The listing builds one solid part. Answer for the finished solid, in the listing's coordinates (mm). A direction names the side the tool comes from. Give positions to 0.01 mm unless a question says otherwise; leave off trailing zeros. Order: outer loops, then holes, each group sorted by start corner. A loop starts at its lowest first (then second) coordinate and runs counter-clockwise, first axis right, second up. Notation, with made-up numbers: (41, 6) - (92, 6) arc R22 cw to (92, 42) - close; hole circle Ø7 at (23, 59.25). An arc over 180 degrees is marked (long way). Write each question's results on one line, items separated by ' | '. Start each with the question number.
1. Which of the six approach directions +Z, -Z, +X, -X, +Y, -Y give full straight-line access (tool end or side, diameter ignored) to faces 5 (the face through (-6, -16.5, 0)), 6 (the face through (-6, 16.5, 0)), 7 (the face through (-430, 0.1, 16.4)), 8 (the face through (-6, 0, -16)), 9 (the face through (-440, 17.5, 0))?
2. Determine the mould class of faces 1 (the face through (440, 0, -17)), 2 (the face through (-6, 0, 16)), 3 (the face through (430, 0.1, 16.4)), 4 (the face through (-450, 0, 0)) for opening direction X: released by +X, released by -X, zero draft, split by the parting line, or undercut.
3. Find the intervals of material crossed by L1, parallel to Z at x = 400, y = 12.75; L2, parallel to Z at x = -311, y = -13; L3, parallel to Y at x = 29, z = -11, in increasing order.
4. Flat-ended cylindrical pins translate along their axes: pin 1 (6 mm diameter, centred on x = -67.5, z = 0.5, fed in from -Y); pin 2 (8 mm diameter, centred on x = 24.5, y = 10.5, fed in from -Z); pin 3 (1.5 mm diameter, centred on x = 83.5, y = 2, fed in from +Z). Find the tip coordinate at first contact, or state that the pin passes through.
5. Section A-A (z = -10) is taken. Give the vertices of the cut face in (x, y), and give its area (3 significant figures).
6. Section B-B (x = -164) is taken. Give the vertices of the cut face in (y, z), and give its area (3 significant figures).
from build123d import *

# Parameters (mm, degrees)
SKETCH_1_W                  = 900
SKETCH_1_H                  = 33
EXTRUDE_1_DEPTH             = 16
SKETCH_2_W                  = 34
SKETCH_2_H                  = 35
EXTRUDE_2_DEPTH             = 20
HOLE_WIZARD_4_5_4_5_1_D     = 4.5
HOLE_WIZARD_4_5_4_5_1_DEPTH = 10
HOLE_WIZARD_4_5_4_5_1_TIP   = 1.351936393


with BuildPart() as part:
    # 草图1 → 凸台-拉伸1 (new, symmetric)
    with BuildSketch(Plane.XY):
        Rectangle(SKETCH_1_W, SKETCH_1_H)
    extrude(amount=EXTRUDE_1_DEPTH, both=True)

    # 草图2 → 凸台-拉伸2 (add)
    with BuildSketch(Plane(origin=(450, 0, 0), x_dir=(0, 0, -1), z_dir=(1, 0, 0))):
        Rectangle(SKETCH_2_W, SKETCH_2_H)
    extrude_2 = extrude(amount=-EXTRUDE_2_DEPTH)

    # 镜向2: 凸台-拉伸2 across plane
    add(extrude_2.mirror(Plane(origin=(0, 0, 0), x_dir=(0, 0, 1), z_dir=(1, 0, 0))))

    # Ø4.5 (4.5) 直径孔1
    with Locations(Plane(origin=(0, 16.5, 0), x_dir=(1, 0, 0), z_dir=(0, 1, 0))):
        with Locations((-400, 0), (400, 0)):
            Hole(HOLE_WIZARD_4_5_4_5_1_D / 2, depth=HOLE_WIZARD_4_5_4_5_1_DEPTH)
            with Locations((0, 0, -(HOLE_WIZARD_4_5_4_5_1_DEPTH + HOLE_WIZARD_4_5_4_5_1_TIP / 2))):  # 118° drill point
                Cone(0, HOLE_WIZARD_4_5_4_5_1_D / 2, HOLE_WIZARD_4_5_4_5_1_TIP, mode=Mode.SUBTRACT)


solid = part.part
Reported:
1) face 5: +Z, -Z, -Y | face 6: +Z, -Z, +Y | face 7: none | face 8: -Z, +Y, -Y | face 9: +Z, -Z, +X, -X, +Y
2) face 1: zero draft | face 2: undercut | face 3: undercut | face 4: released by -X
3) L1: -16 to -2.25, 2.25 to 16 | L2: -16 to 16 | L3: -16.5 to 16.5
4) pin 1: y = -16.5 | pin 2: z = -16 | pin 3: z = 16
5) outline: (-450, -17.5) - (-430, -17.5) - (-430, -16.5) - (430, -16.5) - (430, -17.5) - (450, -17.5) - (450, 17.5) - (430, 17.5) - (430, 16.5) - (-430, 16.5) - (-430, 17.5) - (-450, 17.5) - close | area: 29,800 mm²
6) outline: (-16.5, -16) - (16.5, -16) - (16.5, 16) - (-16.5, 16) - close | area: 1,060 mm²
